The listing builds one solid part. Answer for the finished solid, in the listing's coordinates (mm). A direction names the side the tool comes from. Round coordinates to 2 decimals unless told otherwise and drop trailing zeros. Write each loop counter-clockwise with the first axis right and the second up, starting at its lowest first coordinate (ties: lowest second). Pieces come first, ordered by that corner, then holes. Notation, with made-up numbers: (76.5, 22.5) - (90.5, 22.5) arc R9 ccw to (90.5, 34.5) - close; hole circle Ø6 at (77.5, -37.75). An arc over 180 degrees is marked (long way). Answer in a Markdown table with one row per item.
from build123d import *

# Parameters (mm, degrees)
SKETCH1_W                                           = 160
SKETCH1_H                                           = 100
SKETCH1_R                                           = 35
BOSS_EXTRUDE1_DEPTH                                 = 20
FILLET1_R                                           = 5
HOLE_SPEC_PER_SOCKET_HEAD_CAP_SCREW_TYP_D           = 11
HOLE_SPEC_PER_SOCKET_HEAD_CAP_SCREW_TYP_CBORE_D     = 18
HOLE_SPEC_PER_SOCKET_HEAD_CAP_SCREW_TYP_CBORE_DEPTH = 10.5
HOLE_SPEC_PER_SOCKET_HEAD_CAP_SCREW_2_D             = 11
HOLE_SPEC_PER_SOCKET_HEAD_CAP_SCREW_2_CBORE_D       = 18
HOLE_SPEC_PER_SOCKET_HEAD_CAP_SCREW_2_CBORE_DEPTH   = 11
FILLET2_R                                           = 1


with BuildPart() as part:
    # Sketch1 → Boss-Extrude1 (new body)
    with BuildSketch(Plane.XY):
        Rectangle(SKETCH1_W, SKETCH1_H)
        Circle(SKETCH1_R, mode=Mode.SUBTRACT)
    extrude(amount=BOSS_EXTRUDE1_DEPTH)

    # Fillet1
    fillet1_edges = [part.edges().sort_by_distance(p)[0] for p in [
        (-80, 50, 10),
        (80, 50, 10),
        (80, -50, 10),
        (-80, -50, 10),
    ]]
    fillet(fillet1_edges, radius=FILLET1_R)

    # Hole Spec _per socket head cap screw typ (through all)
    with Locations(Plane.XY.offset(20)):
        with Locations((-36, 36), (36, 36), (-36, -36), (36, -36)):
            CounterBoreHole(HOLE_SPEC_PER_SOCKET_HEAD_CAP_SCREW_TYP_D / 2, HOLE_SPEC_PER_SOCKET_HEAD_CAP_SCREW_TYP_CBORE_D / 2, HOLE_SPEC_PER_SOCKET_HEAD_CAP_SCREW_TYP_CBORE_DEPTH)

    # Hole Spec _per socket head cap screw 2 (through all)
    with Locations(Plane(origin=(0, 0, 0), x_dir=(-1, 0, 0), z_dir=(0, 0, -1))):
        with Locations((-63, 36), (63, 36), (-63, -36), (63, -36)):
            CounterBoreHole(HOLE_SPEC_PER_SOCKET_HEAD_CAP_SCREW_2_D / 2, HOLE_SPEC_PER_SOCKET_HEAD_CAP_SCREW_2_CBORE_D / 2, HOLE_SPEC_PER_SOCKET_HEAD_CAP_SCREW_2_CBORE_DEPTH)

    # Fillet2
    fillet2_edges = [part.edges().sort_by_distance(p)[0] for p in [
        (80, 0, 0),
        (80, 0, 20),
        (-80, 0, 0),
        (0, 50, 0),
        (0, -50, 0),
        (78.535533906, 48.535533906, 0),
        (-78.535533906, 48.535533906, 0),
        (-78.535533906, -48.535533906, 0),
        (78.535533906, -48.535533906, 0),
        (0, -50, 20),
        (-80, 0, 20),
        (0, 50, 20),
        (78.535533906, 48.535533906, 20),
        (-78.535533906, 48.535533906, 20),
        (-78.535533906, -48.535533906, 20),
        (78.535533906, -48.535533906, 20),
    ]]
    fillet(fillet2_edges, radius=FILLET2_R)


solid = part.part
(1) For a pull along X with two mould halves and no side action, classify faces 1 (the flat face through (80, -1, 10)), 2 (the flat face through (-1, -50, 10)), 3 (the cylindrical face through (-67.84, 43.59, 5.42)) as pulls with the +X half, pulls with the -X half, needs draft (parallel to the pull), parting line crosses it, or undercut.
Checked values:
| item | result |
|---|---|
| face 1 | pulls with the +X half |
| face 2 | needs draft |
| face 3 | undercut |
(2) For faces 4 (the flat face through (67, 32, 11)), 5 (the flat face through (40, -32, 9.5)), 6 (the cylindrical face through (-31.95, -32.28, 4.68)), determine the directions among +Z, -Z, +X, -X, +Y, -Y from which every point of the face is accessible in a straight line to the end or side of a thin tool.
Checked values:
| item | result |
|---|---|
| face 4 | -Z |
| face 5 | +Z |
| face 6 | +Z, -Z |
(3) Section A-A (x = -63) is taken. Give the vertices of the cut face in (y, z).
Checked values:
| item | result |
|---|---|
| outline | (-50, 1) arc R1 ccw to (-49, 0) - (-45, 0) - (-45, 11) - (-41.5, 11) - (-41.5, 20) - (-49, 20) arc R1 ccw to (-50, 19) - close; (-30.5, 11) - (-27, 11) - (-27, 0) - (27, 0) - (27, 11) - (30.5, 11) - (30.5, 20) - (-30.5, 20) - close; (41.5, 11) - (45, 11) - (45, 0) - (49, 0) arc R1 ccw to (50, 1) - (50, 19) arc R1 ccw to (49, 20) - (41.5, 20) - close |
(4) Section D-D (z = 3.25) is taken. State how many separate pieces and enclosed holes the cut face has, and give its area (3 significant figures).
Checked values:
| item | result |
|---|---|
| separate pieces | 1 |
| enclosed holes | 9 |
| area | 10,700 mm2 |
(5) Section C-C (y = 0) is taken. Give the vertices of the cut face in (x, z).
Checked values:
| item | result |
|---|---|
| outline | (-80, 1) arc R1 ccw to (-79, 0) - (-35, 0) - (-35, 20) - (-79, 20) arc R1 ccw to (-80, 19) - close; (35, 0) - (79, 0) arc R1 ccw to (80, 1) - (80, 19) arc R1 ccw to (79, 20) - (35, 20) - close |
(6) Find the intervals of material crossed by line 1 (Y direction, x = -36, z = 13.5); line 2 (Y direction, x = -36, z = 6.75); line 3 (X direction, y = -29, z = 3.25), in increasing order.
Checked values:
| item | result |
|---|---|
| line 1 | y = -50 to -45, -27 to 27, 45 to 50 |
| line 2 | y = -50 to -41.5, -30.5 to 30.5, 41.5 to 50 |
| line 3 | x = -80 to -68.66, -57.34 to -19.6, 19.6 to 57.34, 68.66 to 80 |
(7) Section B-B (x = 0) is taken. Give the vertices of the cut face in (y, z), and give its area (3 significant figures).
Checked values:
| item | result |
|---|---|
| outline | (-50, 1) arc R1 ccw to (-49, 0) - (-35, 0) - (-35, 20) - (-49, 20) arc R1 ccw to (-50, 19) - close; (35, 0) - (49, 0) arc R1 ccw to (50, 1) - (50, 19) arc R1 ccw to (49, 20) - (35, 20) - close |
| area | 599 mm2 |
(8) Flat-ended cylindrical pins translate along their axes: pin 1 (14.5 mm diameter, centred on x = 36, y = -36, fed in from +Z); pin 2 (1 mm diameter, centred on x = -29.5, y = -33, fed in from -Z); pin 3 (12.5 mm diameter, centred on x = 63, y = 36, fed in from -Z). Find the tip coordinate at first contact, or state that the pin passes through.
Checked values:
| item | result |
|---|---|
| pin 1 | stops at z = 9.5 |
| pin 2 | stops at z = 0 |
| pin 3 | stops at z = 11 |
